Input: part model. Units: mm. Frame: model coordinates. A direction names the side the tool comes from. Give positions to 0.01 mm unless a question says otherwise; leave off trailing zeros. Order: outer loops, then holes, each group sorted by start corner. A loop starts at its lowest first (then second) coordinate and runs counter-clockwise, first axis right, second up. Notation, with made-up numbers: (80, -38) - (130, -38) arc R29 cw to (130, -3) - close; hole circle Ø8 at (34, 33). An arc over 180 degrees is marked (long way). Answer in a Markdown table with one row per item. Add a question column.
from build123d import *

# Parameters (mm, degrees)
PIN_BODY_80MM_DEPTH             = 80
ARROW_NOSE_CUT_DEPTH            = 82.240384046
ARROW_NOSE_CUT_DEPTH_BACK       = 82.240384046
SLOT_AND_STEP_CUT_DEPTH         = 82.240384046
SLOT_AND_STEP_CUT_DEPTH_BACK    = 82.240384046
SPIGOT_PROFILE_10_R             = 5
SPIGOT_10X12_DEPTH              = 12
COUNTERBORED_HOLE_4_D           = 4
COUNTERBORED_HOLE_4_DEPTH       = 100
COUNTERBORED_HOLE_4_CBORE_D     = 10
COUNTERBORED_HOLE_4_CBORE_DEPTH = 4


with BuildPart() as part:
    # Pin Body Profile → Pin Body 80mm (new body)
    with BuildSketch(Plane(origin=(0, 0, 0), x_dir=(0, 0, -1), z_dir=(1, 0, 0))):
        with BuildLine():
            ThreePointArc((-8.485281374, -8.485281374), (-10, 0), (-8.485281374, 8.485281374))
            ThreePointArc((-8.485281374, 8.485281374), (0, 10), (8.485281374, 8.485281374))
            ThreePointArc((8.485281374, 8.485281374), (10, 0), (8.485281374, -8.485281374))
            ThreePointArc((8.485281374, -8.485281374), (0, -10), (-8.485281374, -8.485281374))
        make_face()
    extrude(amount=PIN_BODY_80MM_DEPTH)

    # Arrow Nose Profile 72deg → Arrow Nose Cut (cut, two sides: drawn at the far end of the back side and taken through both)
    with BuildSketch(Plane.XY.offset(-ARROW_NOSE_CUT_DEPTH_BACK)):
        Polygon((0, 10), (0, 0), (13.763819205, 10), align=None)
        Polygon((13.763819205, -10), (0, 0), (0, -10), align=None)
    extrude(amount=ARROW_NOSE_CUT_DEPTH + ARROW_NOSE_CUT_DEPTH_BACK, mode=Mode.SUBTRACT)

    # Slot and Step Profile → Slot and Step Cut (cut, two sides: drawn at the far end of the back side and taken through both)
    with BuildSketch(Plane.XY.offset(-SLOT_AND_STEP_CUT_DEPTH_BACK)):
        with BuildLine():
            Line((72, 10), (59, -3))
            Line((59, -3), (19, -3))
            ThreePointArc((19, -3), (16, 0), (19, 3))
            Line((19, 3), (55, 3))
            Line((55, 3), (62, 10))
            Line((62, 10), (72, 10))
        make_face()
    extrude(amount=SLOT_AND_STEP_CUT_DEPTH + SLOT_AND_STEP_CUT_DEPTH_BACK, mode=Mode.SUBTRACT)

    # Spigot Profile Ø10 → Spigot Ø10x12 (add)
    with BuildSketch(Plane(origin=(80, 0, 0), x_dir=(0, 0, -1), z_dir=(1, 0, 0))):
        Circle(SPIGOT_PROFILE_10_R)
    extrude(amount=SPIGOT_10X12_DEPTH)

    # Counterbored Hole Ø4
    with Locations(Plane(origin=(36.427461815, 9.999980768, -0.030712762), x_dir=(0, 0.001252347692, 0.999999215812), z_dir=(0, 0.999999215812, -0.001252347692))):
        with Locations((0, 0)):
            CounterBoreHole(COUNTERBORED_HOLE_4_D / 2, COUNTERBORED_HOLE_4_CBORE_D / 2, COUNTERBORED_HOLE_4_CBORE_DEPTH, depth=COUNTERBORED_HOLE_4_DEPTH)


solid = part.part
Q1. Section A-A, the plane x = 50. Return loops of the section in (y, z).
Q2. Line query: probe 1 along X at (y, z) = (7, -0.5); probe 2 along Y at (x, z) = (22, 0); probe 3 along Y at (x, z) = (58.5, 7). Output: solid intervals per line, ascending.
Q3. Section B-B, the plane y = -2. Return loops of the section in (x, z).
Q4. Pull-direction query (Y, two-part tool) for faces 5 (the flat face through (66, 4, 0)), 6 (the cylindrical face through (42, 10, 0)), 7 (the flat face through (80, 5, -2)); classes: +Y half, -Y half, draft (parallel to the pull), parting line (faces both ways), or undercut.
Q5. Access query for faces 1 (the cylindrical face through (85.92, -4.88, 1.08)), 2 (the flat face through (6.786, 4.93, -0.14)), 3 (the cylindrical face through (39.44, -3.715, -9.717)), 4 (the flat face through (58, 6, 0)). Directions: +Z, -Z, +X, -X, +Y, -Y. A direction counts if a zero-diameter tool reaches every point of the face in a straight line with its end or side. Return the directions, or none.
Q6. Section D-D, the plane x = 18. Return loops of the section in (y, z).
Q7. Section C-C, the plane z = 0. State how many separate pieces and enclosed holes the cut face has, then the cut area to 3 significant figures.
Q8. Contact query for flat-ended pins moving along their axis: P1, Ø1, axis at x = 58, z = -5.5, coming from the +Y side; P2, Ø1.5, axis at x = 18.5, y = 5.5, coming from the -Z side; P3, Ø1, axis at x = 46, z = 7.5, coming from the -Y side; P4, Ø6, axis at x = 38.5, z = -0.5, coming from the -Y side. Output: stop coordinate, or through.
Computed:
| question | item | result |
|---|---|---|
| 1 | outline | (-8.49, -8.49) arc R24.52 ccw to (-3, -9.82) - (-3, 9.82) arc R24.52 ccw to (-8.49, 8.49) arc R24.52 ccw to start; (3, -9.82) arc R24.52 ccw to (8.49, -8.49) arc R24.52 ccw to (8.49, 8.49) arc R24.52 ccw to (3, 9.82) - close |
| 2 | probe 1 | x = 9.63 to 31.45, 41.41 to 59, 69 to 80 |
| 2 | probe 2 | y = -10 to -3, 3 to 10 |
| 2 | probe 3 | y = -8.98 to -3, 6.5 to 8.98 |
| 3 | outline | (2.75, -9.92) - (16.76, -9.92) - (16.76, 9.92) - (2.75, 9.92) - close; (60, -9.92) - (80, -9.92) - (80, -4.58) - (92, -4.58) - (92, 4.58) - (80, 4.58) - (80, 9.92) - (60, 9.92) - close |
| 4 | face 5 | undercut |
| 4 | face 6 | +Y half |
| 4 | face 7 | draft |
| 5 | face 1 | +X |
| 5 | face 2 | +Z, -Z, -X, +Y |
| 5 | face 3 | -Z, +X, -X |
| 5 | face 4 | +Z, -Z |
| 6 | outline | (-8.49, -8.49) arc R24.52 ccw to (-2.83, -9.84) - (-2.83, 9.84) arc R24.52 ccw to (-8.49, 8.49) arc R24.52 ccw to start; (2.83, -9.84) arc R24.52 ccw to (8.49, -8.49) arc R24.52 ccw to (8.49, 8.49) arc R24.52 ccw to (2.83, 9.84) - close |
| 7 | separate pieces | 3 |
| 7 | enclosed holes | 0 |
| 7 | area | 1,160 mm^2 |
| 8 | P1 | stops at y = 9.48 |
| 8 | P2 | stops at z = -9.54 |
| 8 | P3 | stops at y = -8.98 |
| 8 | P4 | stops at y = -10 |
